```python
from build123d import *

# Parameters (mm, degrees)
SKETCH1_R           = 15
BOSS_EXTRUDE1_DEPTH = 3
SKETCH3_R           = 3
BOSS_EXTRUDE2_DEPTH = 55
SKETCH4_R           = 3
SKETCH4_W           = 4
SKETCH4_H           = 4
CUT_EXTRUDE1_DEPTH  = 5


with BuildPart() as part:
    # Sketch1 → Boss-Extrude1 (new, symmetric)
    with BuildSketch(Plane(origin=(0, 0, 0), x_dir=(1, 0, 0), z_dir=(0, 1, 0))):
        with Locations(Location((0, 0, 0), (0, 0, 270))):
            Circle(SKETCH1_R)
    extrude(amount=BOSS_EXTRUDE1_DEPTH, both=True)

    # Sketch3 → Boss-Extrude2 (add, symmetric)
    with BuildSketch(Plane(origin=(0, 0, 0), x_dir=(1, 0, 0), z_dir=(0, 1, 0))):
        with Locations(Location((0, -6, 0), (0, 0, 270))):
            Circle(SKETCH3_R)
    extrude(amount=BOSS_EXTRUDE2_DEPTH, both=True)

    # Sketch4 → Cut-Extrude1 (cut)
    with BuildSketch(Plane(origin=(0, 55, 0), x_dir=(1, 0, 0), z_dir=(0, 1, 0))):
        with Locations(Location((0, -6, 0), (0, 0, 270))):
            Circle(SKETCH4_R)
        with Locations((0, -6)):
            Rectangle(SKETCH4_W, SKETCH4_H, mode=Mode.SUBTRACT)
    extrude(amount=-CUT_EXTRUDE1_DEPTH, mode=Mode.SUBTRACT)


solid = part.part
```
Here's how the part is built. I have some questions about the finished solid (model axes, mm). A direction names the side the tool comes from. Round coordinates to 2 decimals unless told otherwise and drop trailing zeros. Order: outer loops, then holes, each group sorted by start corner. A loop starts at its lowest first (then second) coordinate and runs counter-clockwise, first axis right, second up. Notation, with made-up numbers: (45, 13.5) -> (51, 13.5) arc R5 ccw to (51, 22.5) -> close; hole circle Ø8 at (-4, 14.5). An arc over 180 degrees is marked (long way). Use a Markdown table: item, result. Add a question column.
(1) Suppose I cut it at C-C, the plane y = 9. Please give me the cut outline in (x, z), and give its area (3 significant figures).
(2) For faces 1 (the face through (2, 53, 6)), 2 (the face through (-1.15, -28.64, 8.77)), 3 (the face through (-1.15, 26.83, 8.77)), 4 (the face through (0, 53, 4)), which set-ups out of +Z, -Z, +X, -X, +Y, -Y let a thin tool reach every point of the face, with its end or its side?
(3) I need wall thicknesses on line 1 along Y through (x, z) = (9.75, -2.5); line 2 along X through (y, z) = (1.5, -9.75); line 3 along Z through (x, y) = (1.75, -43.5). Which ranges of each line are inside material? Lowest first, please.
(4) Suppose I cut it at A-A, the plane x = 0. Please give me the cut outline in (y, z), and give its area (3 significant figures).
(5) Suppose I cut it at D-D, the plane z = 0. Please give me the cut outline in (x, y), and give its area (3 significant figures).
(6) For pin 1 Ø3 at (y, z) = (52, 7) entering from -X; pin 2 Ø1.5 at (x, y) = (9.5, -4) entering from +Z; pin 3 Ø1.5 at (y, z) = (-1.5, 7) entering from +X; pin 4 Ø12 at (x, y) = (6, -17) entering from +Z, each with a flat end and sliding along its axis, tell me the tip position at first contact or that it passes through.
(7) Suppose I cut it at B-B, the plane z = 6. Please give me the cut outline in (x, y), and give its area (3 significant figures).
Verdict:
| question | item | result |
|---|---|---|
| 1 | outline | circle Ø6 at (0, 6) |
| 1 | area | 28.3 mm2 |
| 2 | face 1 | +Z, -Z, +X, +Y |
| 2 | face 2 | -Y |
| 2 | face 3 | +Y |
| 2 | face 4 | -Z, +X, -X, +Y |
| 3 | line 1 | -3 to 3 |
| 3 | line 2 | -11.4 to 11.4 |
| 3 | line 3 | 3.56 to 8.44 |
| 4 | outline | (-55, 3) -> (-3, 3) -> (-3, -15) -> (3, -15) -> (3, 3) -> (50, 3) -> (50, 4) -> (55, 4) -> (55, 8) -> (50, 8) -> (50, 9) -> (3, 9) -> (3, 15) -> (-3, 15) -> (-3, 9) -> (-55, 9) -> close |
| 4 | area | 794 mm2 |
| 5 | outline | (-15, -3) -> (15, -3) -> (15, 3) -> (-15, 3) -> close |
| 5 | area | 180 mm2 |
| 6 | pin 1 | x = -2 |
| 6 | pin 2 | through |
| 6 | pin 3 | x = 13.64 |
| 6 | pin 4 | z = 9 |
| 7 | outline | (-13.75, -3) -> (-3, -3) -> (-3, -55) -> (3, -55) -> (3, -3) -> (13.75, -3) -> (13.75, 3) -> (3, 3) -> (3, 50) -> (2, 50) -> (2, 55) -> (-2, 55) -> (-2, 50) -> (-3, 50) -> (-3, 3) -> (-13.75, 3) -> close |
| 7 | area | 779 mm2 |
